Source: CAD feature listing. Evaluate the final solid. Frame: model axes, mm. A direction names the side the tool comes from. Round coordinates to 2 decimals unless told otherwise and drop trailing zeros. Loops run counter-clockwise (first coordinate to the right, second up) from the corner with the lowest first, then second, coordinate; pieces in that order, holes last. Notation, with made-up numbers: M 45.25,4.25 L 100.25,4.25 A25 cw 100.25,17.25 Z; hole C -18.75,87.25 d9. An arc over 180 degrees is marked long. One line per item, written item: value.
from build123d import *
from OCP.BRepFilletAPI import BRepFilletAPI_MakeChamfer

# Parameters (mm, degrees)
SKETCH_1_R              = 22.5
EXTRUDE_1_DEPTH         = 900
SKETCH_2_R              = 20
EXTRUDE_2_DEPTH         = 78
SKETCH_3_R              = 17.5
EXTRUDE_3_DEPTH         = 137
EXTRUDE_START           = 48.5
SKETCH_4_R              = 20
EXTRUDE_4_DEPTH         = 48.5
CHAMFER_1_SIZE          = 1.5
CHAMFER_1_SIZE2         = 0.401923789
CUT_EXTRUDE_1_DEPTH     = 5
HOLE_WIZARD_M12_1_D     = 10.2
HOLE_WIZARD_M12_1_DEPTH = 29.25
HOLE_WIZARD_M12_1_TIP   = 3.064389157
HOLE_WIZARD_M10_1_D     = 8.5
HOLE_WIZARD_M10_1_DEPTH = 24.5
HOLE_WIZARD_M10_1_TIP   = 2.553657631
CHAMFER_2_SIZE          = 1.5
CHAMFER_2_SIZE2         = 0.401923789
FILLET_1_R              = 1


with BuildPart() as part:
    # 草图1 → 凸台-拉伸1 (new body)
    with BuildSketch(Plane.XY):
        Circle(SKETCH_1_R)
    extrude(amount=EXTRUDE_1_DEPTH)

    # 草图2 → 凸台-拉伸2 (add)
    with BuildSketch(Plane.XY.offset(900)):
        Circle(SKETCH_2_R)
    extrude(amount=EXTRUDE_2_DEPTH)

    # 草图3 → 凸台-拉伸3 (add)
    with BuildSketch(Plane.XY.offset(978)):
        Circle(SKETCH_3_R)
    extrude(amount=EXTRUDE_3_DEPTH)

    # 草图4 → 凸台-拉伸4 (add)
    with BuildSketch(Plane(origin=(0, 0, 0), x_dir=(-1, 0, 0), z_dir=(0, 0, -1)).offset(EXTRUDE_START)):
        with Locations(Location((0, 0, 0), (0, 0, 180))):
            Circle(SKETCH_4_R)
    extrude(amount=-EXTRUDE_4_DEPTH)

    # 倒角1: one chamfer whose edges measure the first distance from different faces: ONE call of the kernel's chamfer builder (chamfer() names one face for all edges)
    chamfer_1_edges_1 = [part.edges().sort_by_distance(p)[0] for p in [
        (-17.5, 0, 1115),
    ]]
    chamfer_1_side_1 = [part.faces().sort_by_distance(p)[0] for p in [
        (-17.5, 0, 1046.5),
    ]]
    chamfer_1_edges_2 = [part.edges().sort_by_distance(p)[0] for p in [
        (-20, 0, -48.5),
    ]]
    chamfer_1_side_2 = [part.faces().sort_by_distance(p)[0] for p in [
        (-20, 0, -24.25),
    ]]
    chamfer_1_edges_3 = [part.edges().sort_by_distance(p)[0] for p in [
        (-22.5, 0, 900),
    ]]
    chamfer_1_side_3 = [part.faces().sort_by_distance(p)[0] for p in [
        (-22.5, 0, 450),
    ]]
    chamfer_1_edges_4 = [part.edges().sort_by_distance(p)[0] for p in [
        (-20, 0, 978),
    ]]
    chamfer_1_side_4 = [part.faces().sort_by_distance(p)[0] for p in [
        (-20, 0, 939),
    ]]
    chamfer_1 = BRepFilletAPI_MakeChamfer(part.part.solid().wrapped)
    for e in chamfer_1_edges_1:
        chamfer_1.Add(CHAMFER_1_SIZE, CHAMFER_1_SIZE2, e.wrapped, chamfer_1_side_1[0].wrapped)  # the first distance lies on this face
    for e in chamfer_1_edges_2:
        chamfer_1.Add(CHAMFER_1_SIZE, CHAMFER_1_SIZE2, e.wrapped, chamfer_1_side_2[0].wrapped)  # the first distance lies on this face
    for e in chamfer_1_edges_3:
        chamfer_1.Add(CHAMFER_1_SIZE, CHAMFER_1_SIZE2, e.wrapped, chamfer_1_side_3[0].wrapped)  # the first distance lies on this face
    for e in chamfer_1_edges_4:
        chamfer_1.Add(CHAMFER_1_SIZE, CHAMFER_1_SIZE2, e.wrapped, chamfer_1_side_4[0].wrapped)  # the first distance lies on this face
    add(Compound.cast(chamfer_1.Shape()), mode=Mode.REPLACE)

    # 草图5 → 切除-拉伸1 (cut)
    with BuildSketch(Plane(origin=(0, 17.5, 0), x_dir=(1, 0, 0), z_dir=(0, 1, 0))):
        with BuildLine():
            Line((5, -1003), (5, -1073))
            ThreePointArc((5, -1073), (0, -1078), (-5, -1073))
            Line((-5, -1073), (-5, -1003))
            ThreePointArc((-5, -1003), (0, -998), (5, -1003))
        make_face()
    extrude(amount=-CUT_EXTRUDE_1_DEPTH, mode=Mode.SUBTRACT)

    # M12 螺纹孔1
    with Locations(Plane.XY.offset(1115)):
        with Locations((0, 0)):
            Hole(HOLE_WIZARD_M12_1_D / 2, depth=HOLE_WIZARD_M12_1_DEPTH)
            with Locations((0, 0, -(HOLE_WIZARD_M12_1_DEPTH + HOLE_WIZARD_M12_1_TIP / 2))):  # 118° drill point
                Cone(0, HOLE_WIZARD_M12_1_D / 2, HOLE_WIZARD_M12_1_TIP, mode=Mode.SUBTRACT)

    # M10 螺纹孔1
    with Locations(Plane(origin=(0, 0, -48.5), x_dir=(-1, 0, 0), z_dir=(0, 0, -1))):
        with Locations((0, 0)):
            Hole(HOLE_WIZARD_M10_1_D / 2, depth=HOLE_WIZARD_M10_1_DEPTH)
            with Locations((0, 0, -(HOLE_WIZARD_M10_1_DEPTH + HOLE_WIZARD_M10_1_TIP / 2))):  # 118° drill point
                Cone(0, HOLE_WIZARD_M10_1_D / 2, HOLE_WIZARD_M10_1_TIP, mode=Mode.SUBTRACT)

    # 倒角2
    chamfer_2_edges = [part.edges().sort_by_distance(p)[0] for p in [
        (-22.5, 0, 0),
    ]]
    chamfer_2_side = [part.faces().sort_by_distance(p)[0] for p in [
        (-22.5, 0, 449.25),
    ]]
    chamfer(chamfer_2_edges, length=CHAMFER_2_SIZE, length2=CHAMFER_2_SIZE2, reference=chamfer_2_side[0])

    # 圆角1
    fillet_1_edges = [part.edges().sort_by_distance(p)[0] for p in [
        (-20, 0, 0),
    ]]
    fillet(fillet_1_edges, radius=FILLET_1_R)


solid = part.part
1. Pin query (flat end, axial travel): pin 1 (6 mm diameter, centred on x = -2.5, z = 609, fed in from -Y); pin 2 (3 mm diameter, centred on x = -7, z = 880.5, fed in from -Y); pin 3 (1.5 mm diameter, centred on x = -2, y = -0.5, fed in from +Z); pin 4 (9 mm diameter, centred on x = 0, y = 0, fed in from -Z). Return the tip coordinate at first contact, or that it passes through.
Report:
pin 1: stops at y = -22.5
pin 2: stops at y = -21.82
pin 3: stops at z = 1084.37
pin 4: stops at z = -48.5
2. Ray query, line 1 (Y direction, x = 0, z = -42); line 2 (Y direction, x = 0, z = 1092); line 3 (Z direction, x = -18.5, y = -12). Return the intervals inside material, ascending. Write a range as [from, to].
Report:
line 1: y = [-20, -4.25], [4.25, 20]
line 2: y = [-17.5, -5.1], [5.1, 17.5]
line 3: z = [0, 900]
3. Reachability of faces 1 (the face through (4, 4, 1115)), 2 (the face through (-4.336, -19.524, 937.714)), 3 (the face through (-19.98, -0.88, -24.32)) from +Z, -Z, +X, -X, +Y, -Y: full face, straight path, thin tool, end or side. Return the list, or none.
Report:
face 1: +Z, +X, -X, +Y, -Y
face 2: +Z
face 3: -Z
4. Section query A-A (z = 960). Return the cut outline in (x, y).
Report:
outline: C 0,0 d40
5. Section query B-B (z = 807.5). Return the cut outline in (x, y), and give its area (3 significant figures).
Report:
outline: C 0,0 d45
area: 1,590 mm2
